Check sheet for the modelled part. Datum: model origin and axes. Units: mm. Round coordinates to 2 decimals unless told otherwise and drop trailing zeros. Order: outer loops, then holes, each group sorted by start corner. A loop starts at its lowest first (then second) coordinate and runs counter-clockwise, first axis right, second up.
Q1. Cross-section at A-A on x = 60. Record the cut outline in (y, z), then the cut area to 3 significant figures.
Q2. Depth check by flat-ended pin: P1, Ø7.5, axis at x = -58, z = 58.5, coming from the +Y side; P2, Ø6, axis at x = 50, y = 8, coming from the +Z side. Enter the tip coordinate at first touch or a pass-through.
Q3. Scan lines: probe 1 along X at (y, z) = (8, 69); probe 2 along Z at (x, y) = (60, 9.25); probe 3 along Z at (x, y) = (-60, 5). Record each from-to range of solid material in increasing order.
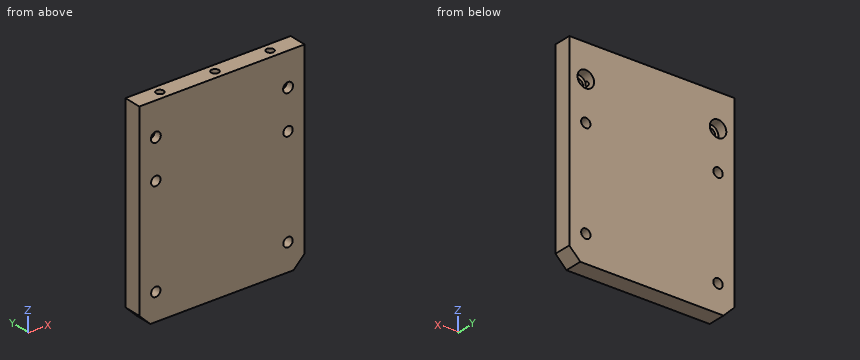
from build123d import *

# Parameters (mm, degrees)
SKETCH_1_W                = 150
SKETCH_1_H                = 180
EXTRUDE_1_DEPTH           = 16
HOLE_WIZARD_M8_1_D        = 6.8
HOLE_WIZARD_M8_1_DEPTH    = 29.25
HOLE_WIZARD_M8_1_TIP      = 2.042926105
HOLE_WIZARD_1_D           = 9
HOLE_WIZARD_1_DEPTH       = 29.25
HOLE_WIZARD_1_CBORE_D     = 15
HOLE_WIZARD_1_CBORE_DEPTH = 9
HOLE_WIZARD_1_TIP         = 2.703872786
HOLE_WIZARD_M10_1_D       = 8.5
CHAMFER_1_SIZE            = 10


with BuildPart() as part:
    # 草图1 → 凸台-拉伸1 (new body)
    with BuildSketch(Plane(origin=(0, 0, 0), x_dir=(1, 0, 0), z_dir=(0, 1, 0))):
        Rectangle(SKETCH_1_W, SKETCH_1_H)
    extrude(amount=EXTRUDE_1_DEPTH)

    # M8 螺纹孔1
    with Locations(Plane.XY.offset(90)):
        with Locations((-50, 8), (0, 8), (50, 8)):
            Hole(HOLE_WIZARD_M8_1_D / 2, depth=HOLE_WIZARD_M8_1_DEPTH)
            with Locations((0, 0, -(HOLE_WIZARD_M8_1_DEPTH + HOLE_WIZARD_M8_1_TIP / 2))):  # 118° drill point
                Cone(0, HOLE_WIZARD_M8_1_D / 2, HOLE_WIZARD_M8_1_TIP, mode=Mode.SUBTRACT)

    # 打孔尺寸(%根据)内六角圆柱头螺钉的类型1
    with Locations(Plane(origin=(0, 16, 0), x_dir=(1, 0, 0), z_dir=(0, 1, 0))):
        with Locations((-60, -60), (60, -60)):
            CounterBoreHole(HOLE_WIZARD_1_D / 2, HOLE_WIZARD_1_CBORE_D / 2, HOLE_WIZARD_1_CBORE_DEPTH, depth=HOLE_WIZARD_1_DEPTH)
            with Locations((0, 0, -(HOLE_WIZARD_1_DEPTH + HOLE_WIZARD_1_TIP / 2))):  # 118° drill point
                Cone(0, HOLE_WIZARD_1_D / 2, HOLE_WIZARD_1_TIP, mode=Mode.SUBTRACT)

    # M10 螺纹孔1 (through all)
    with Locations(Plane(origin=(0, 16, 0), x_dir=(1, 0, 0), z_dir=(0, 1, 0))):
        with Locations((-60, 65.51980275), (60, 65.51980275), (-60, -24.48019725), (60, -24.48019725)):
            Hole(HOLE_WIZARD_M10_1_D / 2)

    # 倒角1
    chamfer_1_edges = [part.edges().sort_by_distance(p)[0] for p in [
        (-75, 8, -90),
        (75, 8, -90),
    ]]
    chamfer(chamfer_1_edges, length=CHAMFER_1_SIZE)


solid = part.part
Results found:
1. outline: (0, -90) - (16, -90) - (16, -69.77) - (0, -69.77) - close; (0, -61.27) - (16, -61.27) - (16, 20.23) - (0, 20.23) - close; (0, 28.73) - (16, 28.73) - (16, 52.5) - (7, 52.5) - (7, 55.5) - (0, 55.5) - close; (0, 64.5) - (7, 64.5) - (7, 67.5) - (16, 67.5) - (16, 90) - (0, 90) - close
1. area: 2,410 mm2
2. P1: stops at y = 7
2. P2: stops at z = 60.51
3. probe 1: x = -75 to -53.4, -46.6 to -3.4, 3.4 to 46.6, 53.4 to 75
3. probe 2: z = -90 to -69.77, -61.27 to 20.23, 28.73 to 52.5, 67.5 to 90
3. probe 3: z = -90 to -69.77, -61.27 to 20.23, 28.73 to 55.5, 64.5 to 90
